from build123d import *

# Parameters (mm, degrees)
BOSS_EXTRUDE1_DEPTH = 2250


with BuildPart() as part:
    # Sketch1 → Boss-Extrude1 (new body)
    with BuildSketch(Plane.XY):
        with BuildLine():
            Line((0, 70), (0, 0))
            Line((0, 0), (70, 0))
            Line((70, 0), (70, 5))
            ThreePointArc((70, 5), (69.121320344, 7.121320344), (67, 8))
            Line((67, 8), (16, 8))
            ThreePointArc((16, 8), (10.343145751, 10.343145751), (8, 16))
            Line((8, 16), (8, 67))
            ThreePointArc((8, 67), (7.121320344, 69.121320344), (5, 70))
            Line((5, 70), (0, 70))
        make_face()
    extrude(amount=BOSS_EXTRUDE1_DEPTH)


solid = part.part
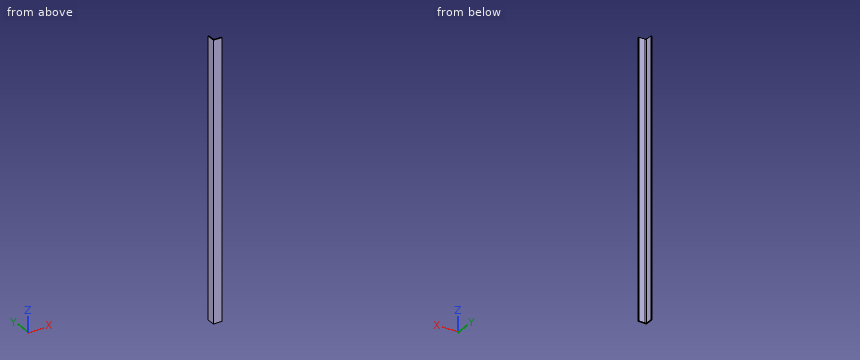
The model under review builds one solid part; all positions refer to its coordinate system, in mm. Give positions to 0.01 mm unless a question says otherwise; leave off trailing zeros. Order: outer loops, then holes, each group sorted by start corner. A loop starts at its lowest first (then second) coordinate and runs counter-clockwise, first axis right, second up. Notation, with made-up numbers: M -38.5,44.5 L -18.5,44.5 A27 cw -18.5,76.5 Z; hole C -15.5,73 d6. An arc over 180 degrees is marked long. Answer in a Markdown table with one row per item. Add a question column.
1. To check wall thickness, follow line 1 along Y through (x, z) = (15.5, 1543); line 2 along X through (y, z) = (25, 1465.5); line 3 along X through (y, z) = (15, 1729). State the ranges of each line that lie inside material, in increasing order.
2. For pin 1 Ø12 at (x, z) = (16.5, 857.5) entering from -Y; pin 2 Ø6 at (y, z) = (53, 723) entering from +X, all flat-tipped, find the tip position at first contact; note any pin that passes through.
3. Add section A-A on z = 1714.5. State the section outline as (x, y) points.
4. Add section B-B on y = 31.5. State the section outline as (x, z) points.
The answers:
| question | item | result |
|---|---|---|
| 1 | line 1 | 0 to 8.02 |
| 1 | line 2 | 0 to 8 |
| 1 | line 3 | 0 to 8.06 |
| 2 | pin 1 | y = 0 |
| 2 | pin 2 | x = 8 |
| 3 | outline | M 0,0 L 70,0 L 70,5 A3 ccw 67,8 L 16,8 A8 cw 8,16 L 8,67 A3 ccw 5,70 L 0,70 Z |
| 4 | outline | M 0,0 L 8,0 L 8,2250 L 0,2250 Z |
